Design review of the part built by this model. Coordinates are the model's own, in mm. Coordinates: 2 decimals unless noted, no trailing zeros. Order: outer loops, then holes, each group sorted by start corner. A loop starts at its lowest first (then second) coordinate and runs counter-clockwise, first axis right, second up. Notation, with made-up numbers: M 30,75.25 L 52,75.25 A30 ccw 52,112.25 Z; hole C 69.5,70 d2. An arc over 180 degrees is marked long. Answer as a JSON object with one key per item and string values.
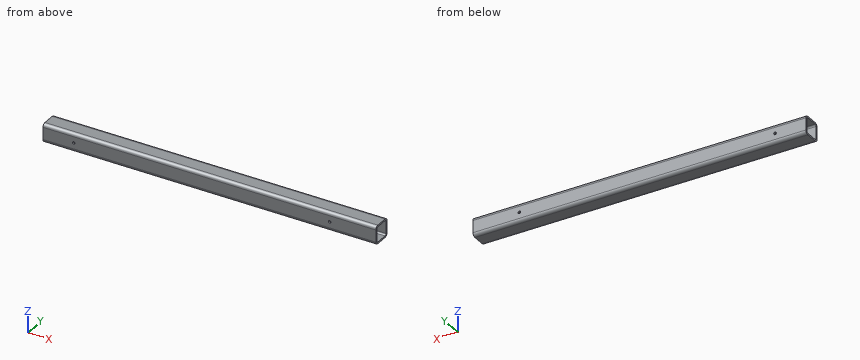
from build123d import *

# Parameters (mm, degrees)
MEMBER_1_DEPTH     = 540
HOLE_WIZARD_M5_1_D = 4.2
HOLE_WIZARD_2_D    = 4.2


with BuildPart() as part:
    # Sketch1 → Member 1 (new body)
    with BuildSketch(Plane(origin=(0, 0, 0), x_dir=(0, 0, -1), z_dir=(1, 0, 0))):
        with BuildLine():
            Line((-9.8, -15), (9.8, -15))
            ThreePointArc((9.8, -15), (13.476955262, -13.476955262), (15, -9.8))
            Line((15, -9.8), (15, 9.8))
            ThreePointArc((15, 9.8), (13.476955262, 13.476955262), (9.8, 15))
            Line((9.8, 15), (-9.8, 15))
            ThreePointArc((-9.8, 15), (-13.476955262, 13.476955262), (-15, 9.8))
            Line((-15, 9.8), (-15, -9.8))
            ThreePointArc((-15, -9.8), (-13.476955262, -13.476955262), (-9.8, -15))
        make_face()
        with BuildLine():
            Line((-9.8, -12.4), (9.8, -12.4))
            ThreePointArc((9.8, -12.4), (11.638477631, -11.638477631), (12.4, -9.8))
            Line((12.4, -9.8), (12.4, 9.8))
            ThreePointArc((12.4, 9.8), (11.638477631, 11.638477631), (9.8, 12.4))
            Line((9.8, 12.4), (-9.8, 12.4))
            ThreePointArc((-9.8, 12.4), (-11.638477631, 11.638477631), (-12.4, 9.8))
            Line((-12.4, 9.8), (-12.4, -9.8))
            ThreePointArc((-12.4, -9.8), (-11.638477631, -11.638477631), (-9.8, -12.4))
        make_face(mode=Mode.SUBTRACT)
    extrude(amount=MEMBER_1_DEPTH)

    # M5 螺纹孔1 (through all)
    with Locations(Plane(origin=(0, -15, 0), x_dir=(-1, 0, 0), z_dir=(0, -1, 0))):
        with Locations((-465, 0)):
            Hole(HOLE_WIZARD_M5_1_D / 2)

    # Hole Wizard 2 (through all)
    with Locations(Plane(origin=(0, -15, 0), x_dir=(-1, 0, 0), z_dir=(0, -1, 0))):
        with Locations((-50, 0)):
            Hole(HOLE_WIZARD_2_D / 2)


solid = part.part
1) Add section B-B (x = 226.5). State the section outline as (y, z) points, and give its area (3 significant figures).
Taken from the geometry:
{"outline": "M -15,-9.8 A5.2 ccw -9.8,-15 L 9.8,-15 A5.2 ccw 15,-9.8 L 15,9.8 A5.2 ccw 9.8,15 L -9.8,15 A5.2 ccw -15,9.8 Z; hole M -12.4,-9.8 A2.6 ccw -9.8,-12.4 L 9.8,-12.4 A2.6 ccw 12.4,-9.8 L 12.4,9.8 A2.6 ccw 9.8,12.4 L -9.8,12.4 A2.6 ccw -12.4,9.8 Z", "area": "268 mm2"}
2) Insertion check: pin 1 Ø1 at (y, z) = (11.5, 5.5) entering from -X. The pin has a flat end and moves straight along its axis. Give the tip position at first contact, or say it passes through.
Taken from the geometry:
{"pin 1": "passes through"}
3) Add section A-A (y = -2.25). State the section outline as (x, z) points, and give its area (3 significant figures).
Taken from the geometry:
{"outline": "M 0,-15 L 540,-15 L 540,-12.4 L 0,-12.4 Z; M 0,12.4 L 540,12.4 L 540,15 L 0,15 Z", "area": "2,810 mm2"}
4) To check wall thickness, follow L1, parallel to Z at x = 432, y = 6; L2, parallel to Z at x = 157, y = -10.5. State the ranges of each line that lie inside material, in increasing order.
Taken from the geometry:
{"L1": "z = -15 to -12.4, 12.4 to 15", "L2": "z = -14.95 to -12.3, 12.3 to 14.95"}
